Can you work these out from the model? Positions are in its coordinate system, mm. Give positions to 0.01 mm unless a question says otherwise; leave off trailing zeros. Order: outer loops, then holes, each group sorted by start corner. A loop starts at its lowest first (then second) coordinate and runs counter-clockwise, first axis right, second up.
Item 1: I'm going to push flat-ended pins straight in: pin 1 Ø5 at (y, z) = (102.5, 5) entering from +X; pin 2 Ø2 at (y, z) = (52, 1) entering from +X; pin 3 Ø12.5 at (x, y) = (56.38, 56.38) entering from +Z; pin 4 Ø3 at (x, z) = (74, 4.5) entering from +Y. Where does each tip first touch, or does it pass through?
Item 2: I want a section at C-C, the plane y = 81.5. Write out the boundary of the cut face in (x, z).
Item 3: I want a section at B-B, the plane z = 4.5. Write out the boundary of the cut face in (x, y).
Item 4: I want a section at A-A, the plane x = 62. Write out the boundary of the cut face in (y, z).
Item 5: If I drill on line 1 along X through (y, z) = (55, 7); line 2 along X through (y, z) = (59.5, 3.5); line 3 along Y through (x, z) = (62, 0.5), over which ranges is the centre line in solid material (lowest first)?
Item 6: I want a section at D-D, the plane x = 46.5. Write out the boundary of the cut face in (y, z), then the cut area to 4 significant figures.
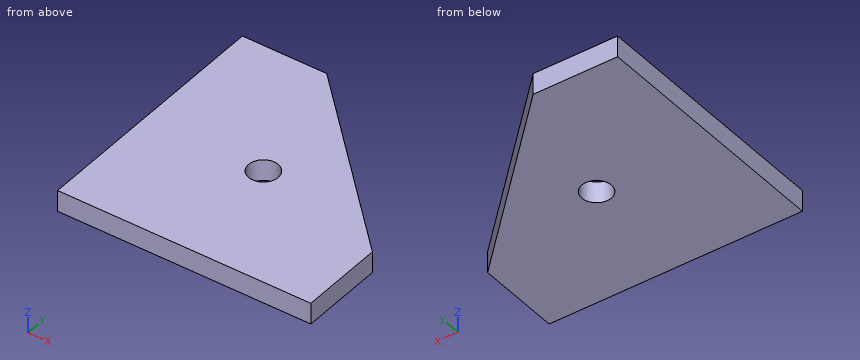
```python
from build123d import *

# Parameters (mm, degrees)
EXTRUDE_1_DEPTH     = 10
HOLE_WIZARD_M16_1_D = 14


with BuildPart() as part:
    # 草图1 → 凸台-拉伸1 (new body)
    with BuildSketch(Plane.XY):
        Polygon((0, 120), (0, 0), (120, 0), (120, 40), (40, 120), align=None)
    extrude(amount=EXTRUDE_1_DEPTH)

    # M16 螺纹孔1 (through all)
    with Locations(Plane(origin=(0, 0, 0), x_dir=(-1, 0, 0), z_dir=(0, 0, -1))):
        with Locations((-56.380361078, 56.380361078)):
            Hole(HOLE_WIZARD_M16_1_D / 2)


solid = part.part
```
Results list:
1. pin 1: stops at x = 60
1. pin 2: stops at x = 109
1. pin 3: passes through
1. pin 4: stops at y = 87.5
2. outline: (0, 0) - (78.5, 0) - (78.5, 10) - (0, 10) - close
3. outline: (0, 0) - (120, 0) - (120, 40) - (40, 120) - (0, 120) - close; hole circle Ø14 at (56.38, 56.38)
4. outline: (0, 0) - (52.21, 0) - (52.21, 10) - (0, 10) - close; (60.55, 0) - (98, 0) - (98, 10) - (60.55, 10) - close
5. line 1: x = 0 to 49.52, 63.24 to 105
5. line 2: x = 0 to 50.11, 62.65 to 100.5
5. line 3: y = 0 to 52.21, 60.55 to 98
6. outline: (0, 0) - (113.5, 0) - (113.5, 10) - (0, 10) - close
6. area: 1,135 mm2
